Part print with two shaded views. Sizes in mm from the minimum x, y, z corner. Round coordinates to 2 decimals unless told otherwise and drop trailing zeros. Order: outer loops, then holes, each group sorted by start corner. A loop starts at its lowest first (then second) coordinate and runs counter-clockwise, first axis right, second up. Notation, with made-up numbers: (88, -8.75) -> (122, -8.75) arc R9 ccw to (122, 3.25) -> close; hole circle Ø10 at (-40, -9.75). An arc over 180 degrees is marked (long way). Put each result on its own line as item: value. Start each with the question number.
Q1. Probe L1, parallel to Y at x = 95, z = 0.4; L2, parallel to X at y = 76, z = 0.45. List the from-to ranges inside material, lowest first.
Q2. Cut at A-A, the plane x = 95. List the corners of the cut face in (y, z).
Q3. Cut at B-B, the plane y = 76. List the corners of the cut face in (x, z), and give its area (3 significant figures).
Q4. Flat gauge pin, fed straight in: P1, Ø2.5, axis at x = 95, y = 4, coming from the +Z side. Where does the tip first touch, or does it go through?
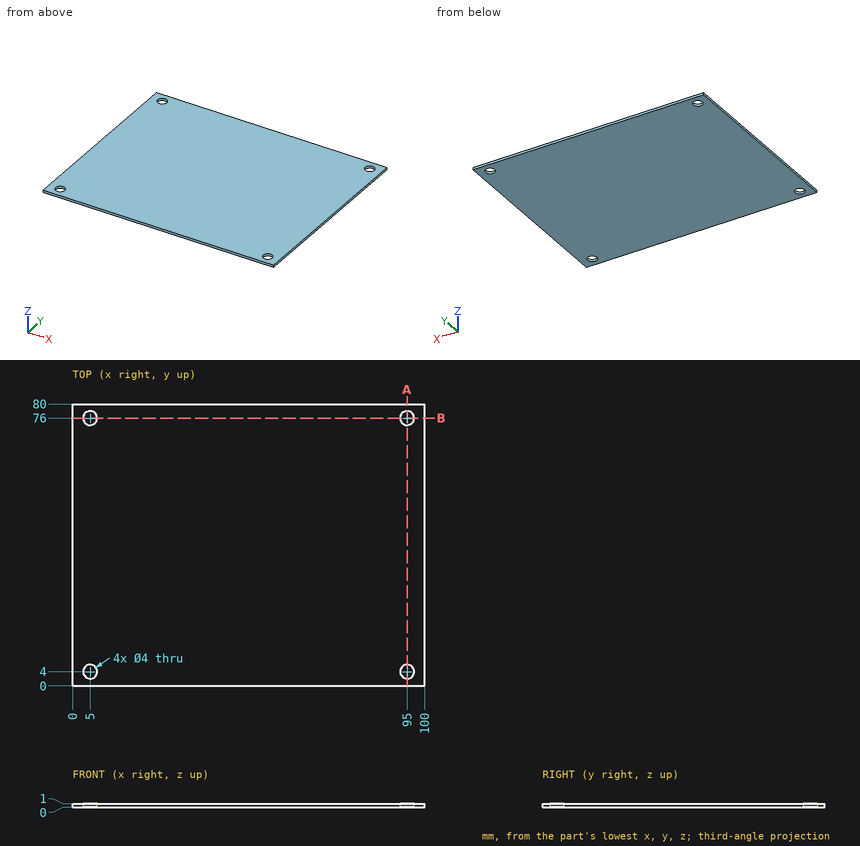
Ans:
1. L1: y = 0 to 2, 6 to 74, 78 to 80
1. L2: x = 0 to 3, 7 to 93, 97 to 100
2. outline: (0, 0) -> (2, 0) -> (2, 1) -> (0, 1) -> close; (6, 0) -> (74, 0) -> (74, 1) -> (6, 1) -> close; (78, 0) -> (80, 0) -> (80, 1) -> (78, 1) -> close
3. outline: (0, 0) -> (3, 0) -> (3, 1) -> (0, 1) -> close; (7, 0) -> (93, 0) -> (93, 1) -> (7, 1) -> close; (97, 0) -> (100, 0) -> (100, 1) -> (97, 1) -> close
3. area: 92.0 mm^2
4. P1: passes through
